Read the model definition and answer for the solid it produces. Units are mm, in the model's axes. Face numbers are marked on the shaded views. A direction names the side the tool comes from. Round coordinates to 2 decimals unless told otherwise and drop trailing zeros. Write each loop counter-clockwise with the first axis right and the second up, starting at its lowest first coordinate (ties: lowest second). Pieces come first, ordered by that corner, then holes.
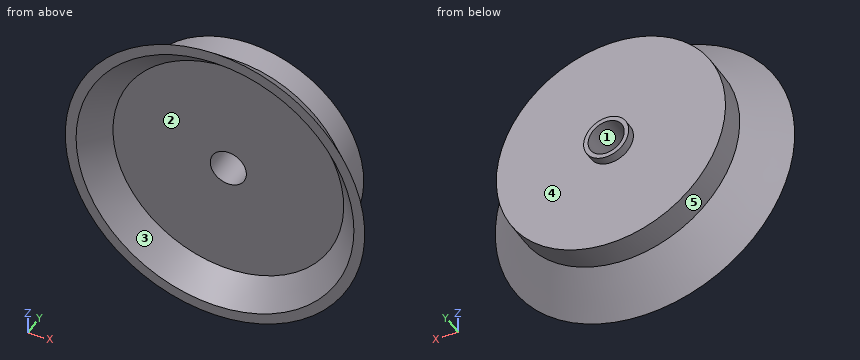
from build123d import *


with BuildPart() as part:
    # 草图1 → 旋转1 (revolve)
    with BuildSketch(Plane.XY, mode=Mode.PRIVATE) as revolve_1_sk:
        Polygon((-6.25, 17.813596491), (-5, 17.813596491), (-5, 4.34498949), (-31.981467322, 4.34498949), (-38.5, -2.686403509), (-41.5, -2.686403509), (-31.765855836, 7.813596491), (-31.765855836, 15.313596491), (-6.25, 15.313596491), align=None)
    revolve(revolve_1_sk.sketch.rotate(Axis((0, 20.559210526, 0), (0, -1, 0)), 270), axis=Axis((0, 20.559210526, 0), (0, -1, 0)))


solid = part.part
Q1. Which of the six approach directions +Z, -Z, +X, -X, +Y, -Y give full straight-line access (tool end or side, diameter ignored) to the marked faces 1 and 2?
Verdict:
face 1: +Y, -Y
face 2: -Y
Q2. Flat-ended cylindrical pins translate along their axes: pin 1 Ø1 at (x, y) = (-26.5, 10) entering from +Z; pin 2 Ø12 at (x, z) = (-4.5, 28.5) entering from -Y; pin 3 Ø8 at (x, z) = (-18.5, 30) entering from +Y. Find the tip coordinate at first contact, or state that the pin passes through.
Verdict:
pin 1: stops at z = 18.25
pin 2: stops at y = 1.25
pin 3: stops at y = 15.31
Q3. Section C-C (y = -0.75) is taken. Determine the outline of the cut face in (x, z).
Verdict:
outline: circle Ø79.41 at (0, 0); hole circle Ø73.41 at (0, 0)
Q4. Straight lines are drawn through the part: probe 1 along X at (y, z) = (14.5, 0); probe 2 along Y at (x, z) = (-18.5, -20); probe 3 along Z at (x, y) = (2, -1.75). For each, find the intervals that lie inside material, in ascending order.
Verdict:
probe 1: x = -31.77 to -5, 5 to 31.77
probe 2: y = 4.34 to 15.31
probe 3: z = -40.58 to -37.58, 37.58 to 40.58
Q5. Section B-B (z = 0) is taken. Determine the outline of the cut face in (x, y), then the cut area to 3 significant figures.
Verdict:
outline: (-41.5, -2.69) - (-38.5, -2.69) - (-31.98, 4.34) - (-5, 4.34) - (-5, 17.81) - (-6.25, 17.81) - (-6.25, 15.31) - (-31.77, 15.31) - (-31.77, 7.81) - close; (5, 4.34) - (31.98, 4.34) - (38.5, -2.69) - (41.5, -2.69) - (31.77, 7.81) - (31.77, 15.31) - (6.25, 15.31) - (6.25, 17.81) - (5, 17.81) - close
area: 647 mm2
Q6. Section D-D (y = 6.5) is taken. Determine the outline of the cut face in (x, z), then the cut area to 3 significant figures.
Verdict:
outline: circle Ø65.97 at (0, 0); hole circle Ø10 at (0, 0)
area: 3,340 mm2
Q7. Determine the mould class of the marked faces 3, 4 and 5 for opening direction Z: pulls with the +Z half, pulls with the -Z half, needs draft (parallel to the pull), parting line crosses it, or undercut.
Verdict:
face 3: undercut
face 4: needs draft
face 5: parting line crosses it
Q8. Section A-A (x = 0) is taken. Determine the outline of the cut face in (y, z), then the cut area to 3 significant figures.
Verdict:
outline: (-2.69, -41.5) - (7.81, -31.77) - (15.31, -31.77) - (15.31, -6.25) - (17.81, -6.25) - (17.81, -5) - (4.34, -5) - (4.34, -31.98) - (-2.69, -38.5) - close; (-2.69, 38.5) - (4.34, 31.98) - (4.34, 5) - (17.81, 5) - (17.81, 6.25) - (15.31, 6.25) - (15.31, 31.77) - (7.81, 31.77) - (-2.69, 41.5) - close
area: 647 mm2
